from build123d import *

# Parameters (mm, degrees)
SKETCH1_W                                           = 8
SKETCH1_H                                           = 8
BOSS_EXTRUDE1_DEPTH                                 = 21
SKETCH2_W                                           = 1.5
SKETCH2_H                                           = 6
CUT_EXTRUDE1_DEPTH                                  = 22.748563171
FILLET1_R                                           = 0.5
CBORE_FOR_M2_HEX_SOCKET_HEAD_CAP_SCREW1_D           = 2.4
CBORE_FOR_M2_HEX_SOCKET_HEAD_CAP_SCREW1_CBORE_D     = 4.4
CBORE_FOR_M2_HEX_SOCKET_HEAD_CAP_SCREW1_CBORE_DEPTH = 2.4
CHAMFER1_SIZE                                       = 0.2
SKETCH7_W                                           = 5
SKETCH7_H                                           = 6.5
CUT_EXTRUDE2_DEPTH                                  = 0.5
FILLET2_R                                           = 0.5


with BuildPart() as part:
    # Sketch1 → Boss-Extrude1 (new body)
    with BuildSketch(Plane.XY):
        Rectangle(SKETCH1_W, SKETCH1_H)
    extrude(amount=BOSS_EXTRUDE1_DEPTH)

    # Sketch2 → Cut-Extrude1 (cut, through all)
    with BuildSketch(Plane.XY.offset(21)):
        with Locations((-3.25, -1)):
            Rectangle(SKETCH2_W, SKETCH2_H)
        with Locations((3.25, -1)):
            Rectangle(SKETCH2_W, SKETCH2_H)
    extrude(amount=-CUT_EXTRUDE1_DEPTH, mode=Mode.SUBTRACT)

    # Fillet1
    fillet1_edges = [part.edges().sort_by_distance(p)[0] for p in [
        (-4, 2, 10.5),
        (4, 2, 10.5),
        (-4, 4, 10.5),
        (4, 4, 10.5),
    ]]
    fillet(fillet1_edges, radius=FILLET1_R)

    # CBORE for M2 Hex Socket Head Cap Screw1 (through all)
    with Locations(Plane(origin=(0, 4, 0), x_dir=(1, 0, 0), z_dir=(0, 1, 0))):
        with Locations((0, -4.5), (0, -16.5)):
            CounterBoreHole(CBORE_FOR_M2_HEX_SOCKET_HEAD_CAP_SCREW1_D / 2, CBORE_FOR_M2_HEX_SOCKET_HEAD_CAP_SCREW1_CBORE_D / 2, CBORE_FOR_M2_HEX_SOCKET_HEAD_CAP_SCREW1_CBORE_DEPTH)

    # Chamfer1
    chamfer1_edges = [part.edges().sort_by_distance(p)[0] for p in [
        (0, -4, 0),
        (0, -4, 21),
        (-3, 2, 0),
        (-2.5, -1, 0),
        (-2.5, -1, 21),
        (-3, 2, 21),
        (2.5, -1, 0),
        (2.5, -1, 21),
        (0, 4, 0),
        (0, 4, 21),
        (-4, 3, 0),
        (4, 3, 0),
        (3, 2, 0),
        (-3.853553391, 2.146446609, 0),
        (-3.853553391, 3.853553391, 0),
        (3.853553391, 2.146446609, 0),
        (3.853553391, 3.853553391, 0),
        (4, 3, 21),
        (3, 2, 21),
        (-4, 3, 21),
        (-3.853553391, 2.146446609, 21),
        (-3.853553391, 3.853553391, 21),
        (3.853553391, 2.146446609, 21),
        (3.853553391, 3.853553391, 21),
    ]]
    chamfer(chamfer1_edges, length=CHAMFER1_SIZE)

    # Sketch7 → Cut-Extrude2 (cut)
    with BuildSketch(Plane(origin=(0, 4, 0), x_dir=(1, 0, 0), z_dir=(0, 1, 0))):
        with Locations((0, -10.5)):
            Rectangle(SKETCH7_W, SKETCH7_H)
    extrude(amount=-CUT_EXTRUDE2_DEPTH, mode=Mode.SUBTRACT)

    # Fillet2
    fillet2_edges = [part.edges().sort_by_distance(p)[0] for p in [
        (2.5, 3.75, 7.25),
        (2.5, 3.75, 13.75),
        (-2.5, 3.75, 13.75),
        (-2.5, 3.75, 7.25),
    ]]
    fillet(fillet2_edges, radius=FILLET2_R)


solid = part.part
Could you check a few things on this model? Use its own coordinates, in mm. A direction names the side the tool comes from. Coordinates: 2 decimals unless noted, no trailing zeros. Order: outer loops, then holes, each group sorted by start corner. A loop starts at its lowest first (then second) coordinate and runs counter-clockwise, first axis right, second up. Notation, with made-up numbers: (-8.75, -15) -> (13.25, -15) arc R22 ccw to (13.25, -6) -> close; hole circle Ø4 at (23, 39.5). An arc over 180 degrees is marked (long way). One line per item, written item: value. Start each with the question number.
1) Imagine slicing it at C-C on z = 4.5. List the corners of the cut face in (x, y) for me, plus the area to 3 significant figures.
2) Imagine slicing it at D-D on z = 1.75. List the corners of the cut face in (x, y) for me.
3) We'd pull the mould along Z, two halves only. Please class faces 6 (the flat face through (0, 1, 21)), 7 (the flat face through (4, 3, 10)), 8 (the flat face through (0, 3.5, 10)): +Z half, -Z half, draft (parallel to the pull), parting line (faces both ways), or undercut.
4) I'm going to push flat-ended pins straight in: pin 1 (0.8 mm diameter, centred on x = 3, z = 8, fed in from -Y); pin 2 (2 mm diameter, centred on x = 0, z = 16.5, fed in from +Y); pin 3 (1.8 mm diameter, centred on y = -0.5, z = 10.5, fed in from -X); pin 4 (2.5 mm diameter, centred on x = 0, z = 4.5, fed in from -Y). Where does each tip first touch, or does it pass through?
5) Imagine slicing it at B-B on y = 0. List the corners of the cut face in (x, z) for me.
6) If I drill on L1, parallel to Z at x = 0, y = 2.95; L2, parallel to X at y = -2.15, z = 4.5; L3, parallel to Z at x = 0, y = 0.4, over which ranges is the centre line in solid material (lowest first)? Write a range as [from, to].
7) Which directions (+Z, -Z, +X, -X, +Y, -Y) give clear straight access to the entire face, cutting with the end or side of a thin tool? Please do faces 1 (the flat face through (-3, 2, 11)), 2 (the flat face through (0, 1.6, 18)), 3 (the flat face through (2.5, -1, 11)), 4 (the flat face through (0, 1, 0)), 5 (the cylindrical face through (0.26, -1.24, 17.67)).
8) Imagine slicing it at A-A on x = 0. List the corners of the cut face in (y, z) for me.
Answer list:
1. outline: (-4, 2.5) arc R0.5 ccw to (-3.5, 2) -> (-2.5, 2) -> (-2.5, -4) -> (-1.2, -4) -> (-1.2, 1.6) -> (-2.2, 1.6) -> (-2.2, 4) -> (-3.5, 4) arc R0.5 ccw to (-4, 3.5) -> close; (1.2, -4) -> (2.5, -4) -> (2.5, 2) -> (3.5, 2) arc R0.5 ccw to (4, 2.5) -> (4, 3.5) arc R0.5 ccw to (3.5, 4) -> (2.2, 4) -> (2.2, 1.6) -> (1.2, 1.6) -> close
1. area: 21.8 mm2
2. outline: (-4, 2.5) arc R0.5 ccw to (-3.5, 2) -> (-2.5, 2) -> (-2.5, -4) -> (2.5, -4) -> (2.5, 2) -> (3.5, 2) arc R0.5 ccw to (4, 2.5) -> (4, 3.5) arc R0.5 ccw to (3.5, 4) -> (-3.5, 4) arc R0.5 ccw to (-4, 3.5) -> close
3. face 6: +Z half
3. face 7: draft
3. face 8: undercut
4. pin 1: stops at y = 2
4. pin 2: passes through
4. pin 3: stops at x = -2.5
4. pin 4: stops at y = -4
5. outline: (-2.5, 0.2) -> (-2.3, 0) -> (2.3, 0) -> (2.5, 0.2) -> (2.5, 20.8) -> (2.3, 21) -> (-2.3, 21) -> (-2.5, 20.8) -> close; hole circle Ø2.4 at (0, 4.5); hole circle Ø2.4 at (0, 16.5)
6. L1: z = [0, 2.3], [6.7, 14.3], [18.7, 21]
6. L2: x = [-2.5, -1.2], [1.2, 2.5]
6. L3: z = [0, 3.3], [5.7, 15.3], [17.7, 21]
7. face 1: +Z, -Z, -X, -Y
7. face 2: +Y
7. face 3: +Z, -Z, +X, -Y
7. face 4: -Z, +X, -X, +Y, -Y
7. face 5: +Y, -Y
8. outline: (-4, 0.2) -> (-3.8, 0) -> (3.8, 0) -> (4, 0.2) -> (4, 2.3) -> (1.6, 2.3) -> (1.6, 3.3) -> (-4, 3.3) -> close; (-4, 5.7) -> (1.6, 5.7) -> (1.6, 6.7) -> (4, 6.7) -> (4, 7.25) -> (3.5, 7.25) -> (3.5, 13.75) -> (4, 13.75) -> (4, 14.3) -> (1.6, 14.3) -> (1.6, 15.3) -> (-4, 15.3) -> close; (-4, 17.7) -> (1.6, 17.7) -> (1.6, 18.7) -> (4, 18.7) -> (4, 20.8) -> (3.8, 21) -> (-3.8, 21) -> (-4, 20.8) -> close
